```python
from build123d import *

# Parameters (mm, degrees)
EXTRUDE_1_DEPTH              = 35
FILLET_1_R                   = 10
SKETCH_2_R                   = 31.5
CUT_EXTRUDE_1_DEPTH          = 13
CUT_EXTRUDE_2_DEPTH          = 103.713192921
CUT_EXTRUDE_2_DEPTH_BACK     = 103.713192921
SKETCH_3_R                   = 20
HOLE_WIZARD_M6_1_D           = 6.6
HOLE_WIZARD_M6_1_CBORE_D     = 11
HOLE_WIZARD_M6_1_CBORE_DEPTH = 6.8
CHAMFER_1_SIZE               = 2
HOLE_WIZARD_M4_1_D           = 4.5
HOLE_WIZARD_M4_1_CBORE_D     = 8
HOLE_WIZARD_M4_1_CBORE_DEPTH = 43.6


with BuildPart() as part:
    # 草图1 → 凸台-拉伸1 (new, symmetric)
    with BuildSketch(Plane(origin=(0, 0, 0), x_dir=(1, 0, 0), z_dir=(0, 1, 0))):
        Polygon((0, 0), (90, 0), (90, 60), (65, 60), (65, 25), (0, 25), align=None)
    extrude(amount=EXTRUDE_1_DEPTH, both=True)

    # 圆角1
    fillet_1_edges = [part.edges().sort_by_distance(p)[0] for p in [
        (65, 0, -25),
    ]]
    fillet(fillet_1_edges, radius=FILLET_1_R)

    # 草图2 → 切除-拉伸1 (cut)
    with BuildSketch(Plane.XY):
        with Locations((32.5, 0)):
            Circle(SKETCH_2_R)
    extrude(amount=-CUT_EXTRUDE_1_DEPTH, mode=Mode.SUBTRACT)

    # 草图3 → 切除-拉伸2 (cut, two sides: drawn at the far end of the back side and taken through both)
    with BuildSketch(Plane(origin=(0, 0, -25), x_dir=(-1, 0, 0), z_dir=(0, 0, -1)).offset(-CUT_EXTRUDE_2_DEPTH_BACK)):
        with Locations((-32.5, 0)):
            Circle(SKETCH_3_R)
    extrude(amount=CUT_EXTRUDE_2_DEPTH + CUT_EXTRUDE_2_DEPTH_BACK, mode=Mode.SUBTRACT)

    # M6 六角圆柱头螺钉的柱形沉头孔1 (through all)
    with Locations(Plane.ZY.offset(-65)):
        with Locations((-48, 26), (-48, -26)):
            CounterBoreHole(HOLE_WIZARD_M6_1_D / 2, HOLE_WIZARD_M6_1_CBORE_D / 2, HOLE_WIZARD_M6_1_CBORE_DEPTH)

    # 倒角1
    chamfer_1_edges = [part.edges().sort_by_distance(p)[0] for p in [
        (90, 0, 0),
        (77.5, 35, -60),
        (0, 35, -12.5),
        (77.5, -35, -60),
        (0, -35, -12.5),
    ]]
    chamfer(chamfer_1_edges, length=CHAMFER_1_SIZE)

    # M4 六角圆柱头螺钉的柱形沉头孔1 (through all)
    with Locations(Plane(origin=(0, 0, -60), x_dir=(-1, 0, 0), z_dir=(0, 0, -1))):
        with Locations((-5.5, 27), (-59.5, 27), (-59.5, -27), (-5.5, -27)):
            CounterBoreHole(HOLE_WIZARD_M4_1_D / 2, HOLE_WIZARD_M4_1_CBORE_D / 2, HOLE_WIZARD_M4_1_CBORE_DEPTH)


solid = part.part
```
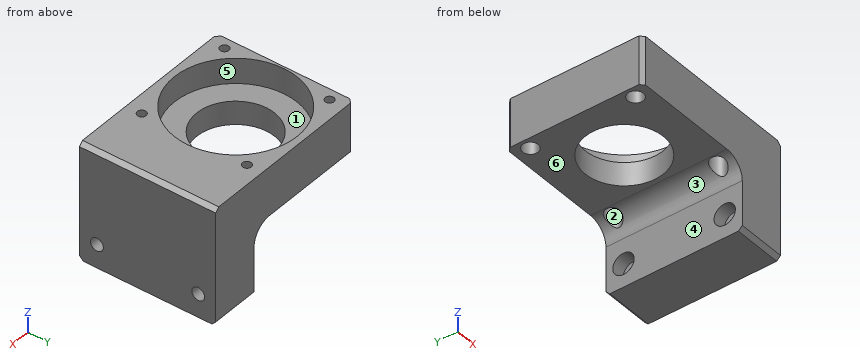
CAD build for the part. Positions are in the model's coordinates, mm. Face numbers are marked on the shaded views. A direction names the side the tool comes from. Coordinates: 2 decimals unless noted, no trailing zeros. Order: outer loops, then holes, each group sorted by start corner. A loop starts at its lowest first (then second) coordinate and runs counter-clockwise, first axis right, second up. Notation, with made-up numbers: M 70.25,36.5 L 96.25,36.5 A31 ccw 96.25,65.5 Z; hole C 51,29 d9. An arc over 180 degrees is marked long. Write each question's results on one line, items separated by ' | '. Start each with the question number.
Q1. Cut at A-A (z = -48). List the corners of the cut face in (x, y).
Q2. Pull direction X, two halves, no side cores. Call the marked faces 4, 5 and 6: +X half, -X half, draft (parallel to the pull), parting line (faces both ways), or undercut.
Q3. Cut at C-C (y = 7). List the corners of the cut face in (x, z) (3 decimals), then the cut area to 3 significant figures.
Q4. Cut at B-B (x = 32.5). List the corners of the cut face in (y, z).
Q5. Drill centre lines: probe 1 along X at (y, z) = (-1, -10); probe 2 along Y at (x, z) = (5.5, -20); probe 3 along Y at (x, z) = (32, -7). Where is each one in solid material? Low to high. Write a range as from..to.
Q6. Cut at D-D (z = -9). List the corners of the cut face in (x, y), then the cut area to 3 significant figures.
Q7. Which spindle directions (+Z, -Z, +X, -X, +Y, -Y) get a long thin tool onto all of the face, cutting with end or side? Do the marked faces 1, 2 and 3. Say none if no direction does.
Q8. Flat gauge pins, fed straight in: P1, Ø7, axis at x = 59.5, y = 27, coming from the -Z side; P2, Ø2, axis at y = -5.5, z = -53, coming from the -X side; P3, Ø9, axis at x = 5.5, y = 27, coming from the +Z side; P4, Ø6.5, axis at x = 61, y = 28, coming from the -Z side. Where does each tip first touch, or does it go through?
Found:
1) outline: M 65,-35 L 90,-35 L 90,-29.3 L 71.8,-29.3 L 71.8,-31.5 L 65,-31.5 Z; M 65,-20.5 L 71.8,-20.5 L 71.8,-22.7 L 90,-22.7 L 90,22.7 L 71.8,22.7 L 71.8,20.5 L 65,20.5 Z; M 65,31.5 L 71.8,31.5 L 71.8,29.3 L 90,29.3 L 90,35 L 65,35 Z
2) face 4: -X half | face 5: undercut | face 6: draft
3) outline: M 0,-25 L 13.765,-25 L 13.765,-13 L 1.788,-13 L 1.788,0 L 0,0 Z; M 51.235,-25 L 55,-25 A10 cw 65,-35 L 65,-60 L 90,-60 L 90,-2 L 88,0 L 63.212,0 L 63.212,-13 L 51.235,-13 Z | area: 1,900 mm²
4) outline: M -35,-25 L -20,-25 L -20,-13 L -31.5,-13 L -31.5,0 L -35,0 Z; M 20,-25 L 35,-25 L 35,0 L 31.5,0 L 31.5,-13 L 20,-13 Z
5) probe 1: 0..1.02, 63.98..90 | probe 2: -35..-31, -23..23, 31..35 | probe 3: -35..-31.5, 31.5..35
6) outline: M 0,-33 L 2,-35 L 90,-35 L 90,35 L 2,35 L 0,33 Z; hole C 32.5,0 d63; hole C 5.5,-27 d4.5; hole C 5.5,27 d4.5; hole C 59.5,-27 d4.5; hole C 59.5,27 d4.5 | area: 3,120 mm²
7) face 1: +Z | face 2: -Z | face 3: -Z, -X, +Y, -Y
8) P1: z = -16.4 | P2: x = 65 | P3: z = 0 | P4: z = -31.2
